Read the model definition and answer for the solid it produces. Units are mm, in the model's axes. Face numbers are marked on the shaded views. A direction names the side the tool comes from. Coordinates: 2 decimals unless noted, no trailing zeros. Loops run counter-clockwise (first coordinate to the right, second up) from the corner with the lowest first, then second, coordinate; pieces in that order, holes last. Notation, with made-up numbers: (73, 2) - (129, 2) arc R13 ccw to (129, 26) - close; hole circle Ø5 at (7, 83). An arc over 180 degrees is marked (long way). One line per question, with ' | ' between items. Start each with the question number.
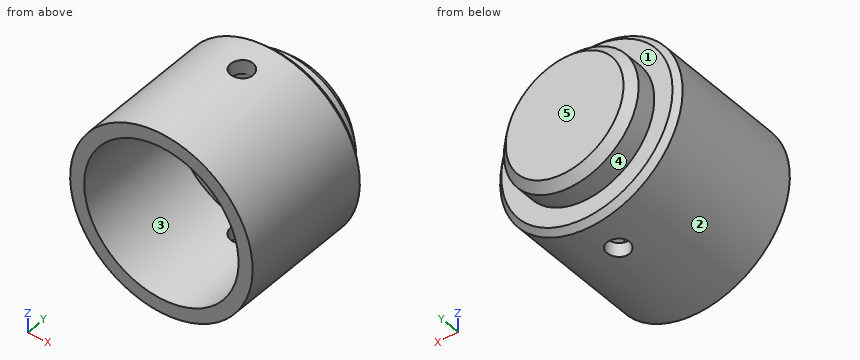
```python
from build123d import *

# Parameters (mm, degrees)
CHAMFER1_SIZE      = 3
CHAMFER2_SIZE      = 2
CUT_EXTRUDE1_START = -20
SKETCH3_R          = 4
CUT_EXTRUDE1_DEPTH = 105
CUT_EXTRUDE2_START = 125
SKETCH4_R          = 4
CUT_EXTRUDE2_DEPTH = 105


with BuildPart() as part:
    # Sketch1 → Revolve1 (revolve)
    with BuildSketch(Plane.XY, mode=Mode.PRIVATE) as revolve1_sk:
        Polygon((0, 60), (-24, 60), (-24, 50), (-32.5, 50), (-32.5, 0), (0, 0), align=None)
    revolve(revolve1_sk.sketch.rotate(Axis((0, 0, 0), (0, 1, 0)), 270), axis=Axis((0, 0, 0), (0, 1, 0)))

    # Chamfer1
    chamfer1_edges = [part.edges().sort_by_distance(p)[0] for p in [
        (0, 60, 24),
    ]]
    chamfer(chamfer1_edges, length=CHAMFER1_SIZE)

    # Chamfer2
    chamfer2_edges = [part.edges().sort_by_distance(p)[0] for p in [
        (0, 50, 32.5),
    ]]
    chamfer(chamfer2_edges, length=CHAMFER2_SIZE)

    # Sketch2 → Cut-Revolve1 (revolve, cut)
    with BuildSketch(Plane.XY):
        Polygon((-27.5, 0), (-27.5, 40), (-15, 40), (-15, 38), (0, 38), (0, 0), align=None)
    revolve(axis=Axis((0, 38, 0), (0, -1, 0)), mode=Mode.SUBTRACT)

    # Sketch3 → Cut-Extrude1 (cut)
    with BuildSketch(Plane.XY.offset(CUT_EXTRUDE1_START)):
        with Locations(Location((0, 36, 0), (0, 0, 90))):
            Circle(SKETCH3_R)
    extrude(amount=-CUT_EXTRUDE1_DEPTH, mode=Mode.SUBTRACT)

    # Sketch4 → Cut-Extrude2 (cut)
    with BuildSketch(Plane.XY.offset(CUT_EXTRUDE2_START)):
        with Locations(Location((0, 36, 0), (0, 0, 90))):
            Circle(SKETCH4_R)
    extrude(amount=-CUT_EXTRUDE2_DEPTH, mode=Mode.SUBTRACT)

    # Sketch7 → Cut-Revolve2 (revolve, cut)
    with BuildSketch(Plane(origin=(0, 0, 0), x_dir=(0, 0, -1), z_dir=(1, 0, 0)), mode=Mode.PRIVATE) as cut_revolve2_sk:
        Polygon((-5.375, 38), (-5.375, 50), (0, 53.103257697), (0, 38), align=None)
    revolve(cut_revolve2_sk.sketch.rotate(Axis((0, 53.103257697, 0), (0, -1, 0)), 180), axis=Axis((0, 53.103257697, 0), (0, -1, 0)), mode=Mode.SUBTRACT)


solid = part.part
```
1) Which of the six approach directions +Z, -Z, +X, -X, +Y, -Y give full straight-line access (tool end or side, diameter ignored) to the marked faces 1 and 2?
2) Find the intervals of material crossed by line 1 along X through (y, z) = (21, 0); line 2 along X through (y, z) = (46, 0) (3 decimals); line 3 along X through (y, z) = (39, 13), in increasing order. Write a range as from..to.
3) Given pin 1 Ø5 at (x, z) = (-18.5, 25) entering from +Y; pin 2 Ø6.5 at (x, y) = (0, 36) entering from +Z; pin 3 Ø9 at (x, z) = (3.5, -1.5) entering from -Y, each flat-ended and moving along its own axis, determine where each tip first touches the part or whether it passes through.
4) The part is cut by section B-B on y = 22. Write down the section's boundary in (x, z), and give its area (3 significant figures).
5) The part is cut by section A-A on y = 36. Write down the section's boundary in (x, z).
6) The mould has two halves that part along Z. Classify the marked faces 3, 4 and 5: released by +Z, released by -Z, zero draft, split by the parting line, or undercut.
7) The part is cut by section C-C on x = -2.5. Count the separate pieces of the cut face and the enclosed holes in it, and give its area (3 significant figures).
Answer below:
1) face 1: +Y | face 2: +Y, -Y
2) line 1: -32.5..-27.5, 27.5..32.5 | line 2: -32.5..-5.375, 5.375..32.5 | line 3: -29.79..-24.23, -7.48..7.48, 24.23..29.79
3) pin 1: y = 50 | pin 2: z = 15 | pin 3: y = 38
4) outline: circle Ø65 at (0, 0); hole circle Ø55 at (0, 0) | area: 942 mm2
5) outline: (-4, -32.25) - (-4, -27.21) arc R27.5 cw to (-4, 27.21) - (-4, 32.25) arc R32.5 ccw to start; (4, -32.25) arc R32.5 ccw to (4, 32.25) - (4, 27.21) arc R27.5 cw to (4, -27.21) - close
6) face 3: undercut | face 4: split by the parting line | face 5: zero draft
7) separate pieces: 3 | enclosed holes: 0 | area: 1,390 mm2
